Read the model definition and answer for the solid it produces. Units are mm, in the model's axes. Face numbers are marked on the shaded views. A direction names the side the tool comes from. Give positions to 0.01 mm unless a question says otherwise; leave off trailing zeros. Order: outer loops, then holes, each group sorted by start corner. A loop starts at its lowest first (then second) coordinate and runs counter-clockwise, first axis right, second up. Notation, with made-up numbers: (12, 78) - (35, 78) arc R21 cw to (35, 98) - close; hole circle Ø8 at (37, 67). An arc over 180 degrees is marked (long way). One line per item, written item: value. Start each with the question number.
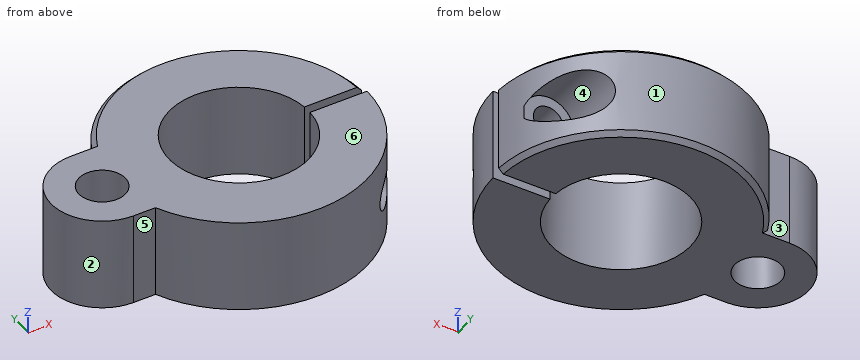
```python
from build123d import *

# Parameters (mm, degrees)
EXTRUDE_1_DEPTH              = 20
CUT_EXTRUDE_1_DEPTH          = 54.265842714
SKETCH_3_W                   = 15
SKETCH_3_H                   = 20
HOLE_WIZARD_10_0_10_1_D      = 10
SKETCH_6_W                   = 2.5
SKETCH_6_H                   = 26.5
HOLE_WIZARD_M6_1_D           = 6.5
HOLE_WIZARD_M6_1_DEPTH       = 50.215633411
HOLE_WIZARD_M6_1_CBORE_D     = 11
HOLE_WIZARD_M6_1_CBORE_DEPTH = 14.715633411
CHAMFER_1_SIZE               = 1


with BuildPart() as part:
    # 草图1 → 凸台-拉伸1 (new body)
    with BuildSketch(Plane.XY.offset(10)):
        with BuildLine():
            Line((-25.204166322, 11), (-30, 11))
            ThreePointArc((-30, 11), (-41, 0), (-30, -11))
            Line((-30, -11), (-25.204166322, -11))
            ThreePointArc((-25.204166322, -11), (27.5, 0), (-25.204166322, 11))
        make_face()
    extrude(amount=-EXTRUDE_1_DEPTH)

    # 草图2 → 切除-拉伸1 (cut, through all)
    with BuildSketch(Plane(origin=(0, 0, -10), x_dir=(-1, 0, 0), z_dir=(0, 0, -1))):
        with BuildLine():
            Line((-27.481812167, -1), (-14.966629547, -1))
            ThreePointArc((-14.966629547, -1), (-15, 0), (-14.966629547, 1))
            Line((-14.966629547, 1), (-27.481812167, 1))
            ThreePointArc((-27.481812167, 1), (-27.5, 0), (-27.481812167, -1))
        make_face()
    extrude(amount=-CUT_EXTRUDE_1_DEPTH, mode=Mode.SUBTRACT)

    # 草图3 → 切除-旋转1 (revolve, cut)
    with BuildSketch(Plane.XZ):
        with Locations((7.5, 0)):
            Rectangle(SKETCH_3_W, SKETCH_3_H)
    revolve(axis=Axis((0, 0, 10), (0, 0, -1)), mode=Mode.SUBTRACT)

    # Ø10.0 (10) 直径孔1 (through all)
    with Locations(Plane.XY.offset(10)):
        with Locations((-30, 0)):
            Hole(HOLE_WIZARD_10_0_10_1_D / 2)

    # 草图6 → Ø5.0 (5) 直径孔1 (revolve, cut)
    with BuildSketch(Plane(origin=(21, -1, 0), x_dir=(0, 0, 1), z_dir=(1, 0, 0))):
        with Locations((1.25, 13.25)):
            Rectangle(SKETCH_6_W, SKETCH_6_H)
    revolve(axis=Axis((21, 5.35, 0), (0, -1, 0)), mode=Mode.SUBTRACT)

    # M6 六角头螺栓的柱形沉头孔1
    with Locations(Plane(origin=(0, 22.715633411, 0), x_dir=(1, 0, 0), z_dir=(0, 1, 0))):
        with Locations((21, 0)):
            CounterBoreHole(HOLE_WIZARD_M6_1_D / 2, HOLE_WIZARD_M6_1_CBORE_D / 2, HOLE_WIZARD_M6_1_CBORE_DEPTH, depth=HOLE_WIZARD_M6_1_DEPTH)

    # 倒角1
    chamfer_1_edges = [part.edges().sort_by_distance(p)[0] for p in [
        (5.128052033, 27.017643908, -10),
        (5.128052033, 27.017643908, 10),
    ]]
    chamfer(chamfer_1_edges, length=CHAMFER_1_SIZE)


solid = part.part
```
1) Section B-B on z = 2.5 is taken. Write down the section's boundary in (x, y).
2) Section C-C on x = 0 is taken. Write down the section's boundary in (y, z).
3) For the marked faces 5 and 6, determine the directions among +Z, -Z, +X, -X, +Y, -Y from which every point of the face is accessible in a straight line to the end or side of a thin tool.
4) The mould has two halves that part along X. Classify the marked faces 1, 2, 3 and 4: +X half, -X half, draft (parallel to the pull), parting line (faces both ways), or undercut.
5) Each of these flat-tipped pins is pushed along its axis until it touches: pin 1 (2 mm diameter, centred on y = -13.5, z = -5, fed in from -X); pin 2 (6 mm diameter, centred on x = -3.5, z = -8, fed in from +Y); pin 3 (5 mm diameter, centred on x = 13.5, z = -7, fed in from -Y); pin 4 (6 mm diameter, centred on x = 21, z = 0, fed in from +Y). Where does it stop, or does it pass through?
6) Find the intervals of material crossed by probe 1 along X at (y, z) = (-4.5, 7.25); probe 2 along X at (y, z) = (6.5, -2.25); probe 3 along Z at (x, y) = (21, -17), in increasing order. Write a range as from..to.
7) Section D-D on y = -10 is taken. Write down the section's boundary in (x, z).
8) Section A-A on y = 0 is taken. Write down the section's boundary in (x, z), plus the area to 3 significant figures.
Solved:
1. outline: (-30, -11) - (-25.2, -11) arc R27.5 ccw to (18.92, -19.95) - (18.92, -1) - (14.97, -1) arc R15 cw (long way) to (14.97, 1) - (18.92, 1) - (18.92, 8) - (16.1, 8) - (16.1, 22.29) arc R27.5 ccw to (-25.2, 11) - (-30, 11) arc R11 ccw to start; (23.08, -14.96) arc R27.5 ccw to (27.48, -1) - (23.08, -1) - close; (23.08, 1) - (27.48, 1) arc R27.5 ccw to (25.9, 9.25) - (25.9, 8) - (23.08, 8) - close; hole circle Ø10 at (-30, 0)
2. outline: (-27.5, -10) - (-15, -10) - (-15, 10) - (-27.5, 10) - close; (15, -10) - (26.5, -10) - (27.5, -9) - (27.5, 9) - (26.5, 10) - (15, 10) - close
3. face 5: +Z, -Z, -X, -Y
3. face 6: +Z, +X, -X, +Y, -Y
4. face 1: parting line
4. face 2: -X half
4. face 3: draft
4. face 4: undercut
5. pin 1: stops at x = -24.49
5. pin 2: stops at y = 27.5
5. pin 3: stops at y = -25.2
5. pin 4: passes through
6. probe 1: x = -40.04..-32.18, -27.82..-14.31, 14.31..27.13
6. probe 2: x = -38.87..-13.52, 13.52..18.65, 23.35..26.72
6. probe 3: z = -10..-3.25, 3.25..10
7. outline: (-34.58, -10) - (-11.18, -10) - (-11.18, 10) - (-34.58, 10) - close; (11.18, -10) - (25.62, -10) - (25.62, 10) - (11.18, 10) - close; hole circle Ø6.5 at (21, 0)
8. outline: (-41, -10) - (-35, -10) - (-35, 10) - (-41, 10) - close; (-25, -10) - (-15, -10) - (-15, 10) - (-25, 10) - close
8. area: 320 mm2
